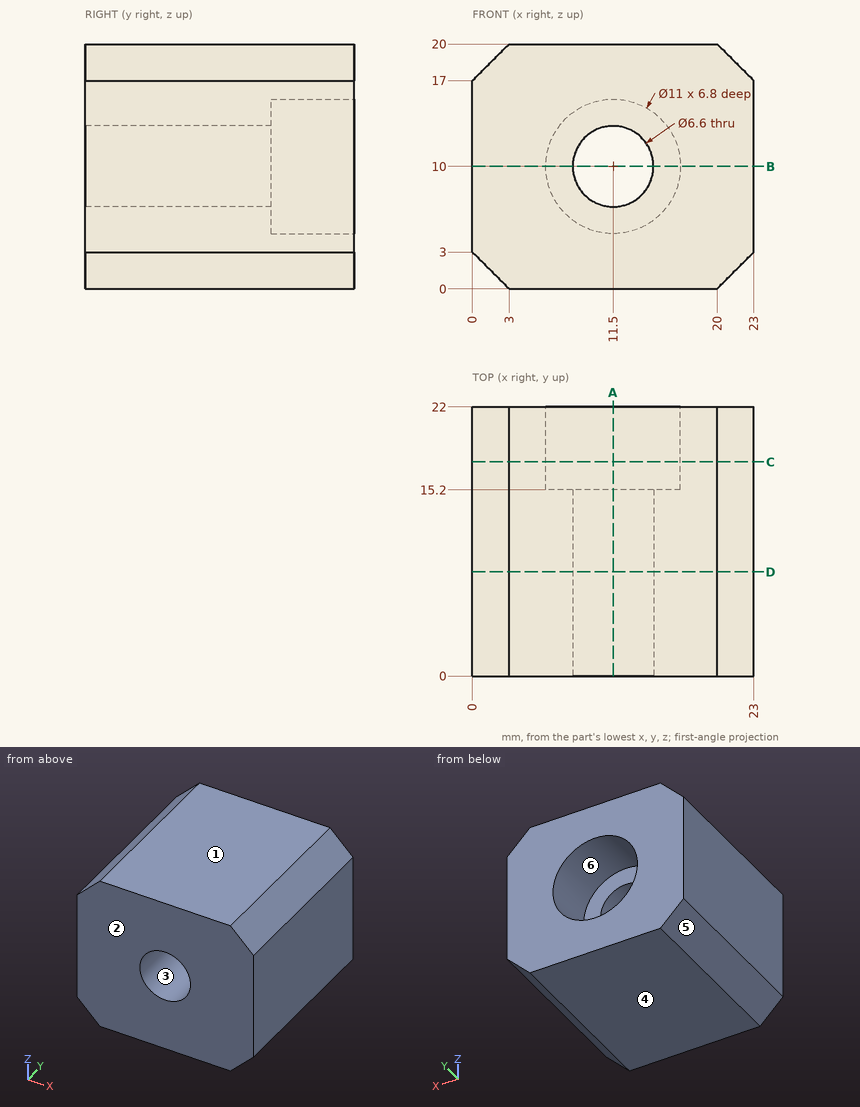
Can you work these out from the drawing? Everything is in mm from the part's minimum corner. A direction names the side the tool comes from. Round coordinates to 2 decimals unless told otherwise and drop trailing zeros. Write each loop counter-clockwise with the first axis right and the second up, starting at its lowest first coordinate (ties: lowest second). Pieces come first, ordered by that corner, then holes. Notation, with made-up numbers: (29.5, -6.5) - (52.5, -6.5) arc R18 ccw to (52.5, 15.5) - close; hole circle Ø5 at (-14, 24.5). An arc over 180 degrees is marked (long way). Put each result on its own line as item: value. Start each with the question number.
(1) I need wall thicknesses on probe 1 along X at (y, z) = (4.75, 10); probe 2 along Z at (x, y) = (11.5, 11.5); probe 3 along Z at (x, y) = (11.5, 16.75). Which ranges of each line are inside material? Lowest first, please.
(2) I want a section at A-A, the plane x = 11.5. Please give me the cut outline in (y, z), plus the area to 3 significant figures.
(3) I want a section at C-C, the plane y = 17.5. Please give me the cut outline in (x, z).
(4) Will these pins go through, and if not, where does the flat tip stop? pin 1 (3.5 mm diameter, centred on x = 13, z = 9, fed in from +Y); pin 2 (5.5 mm diameter, centred on x = 11.5, z = 10, fed in from -Y).
(5) I want a section at D-D, the plane y = 8.5. Please give me the cut outline in (x, z), plus the area to 3 significant figures.
(6) Thinking about a two-plate mould opening in Z: for the marked faces 1, 2, 3 and 4, which applies, released by +Z, released by -Z, zero draft, split by the parting line, or undercut?
(7) I want a section at B-B, the plane z = 10. Please give me the cut outline in (x, y), plus the area to 3 significant figures.
(8) For the marked faces 5 and 6, which set-ups out of +Z, -Z, +X, -X, +Y, -Y let a thin tool reach every point of the face, with its end or its side?
Here are the results:
1. probe 1: x = 0 to 8.2, 14.8 to 23
1. probe 2: z = 0 to 6.7, 13.3 to 20
1. probe 3: z = 0 to 4.5, 15.5 to 20
2. outline: (0, 0) - (22, 0) - (22, 4.5) - (15.2, 4.5) - (15.2, 6.7) - (0, 6.7) - close; (0, 13.3) - (15.2, 13.3) - (15.2, 15.5) - (22, 15.5) - (22, 20) - (0, 20) - close
2. area: 265 mm^2
3. outline: (0, 3) - (3, 0) - (20, 0) - (23, 3) - (23, 17) - (20, 20) - (3, 20) - (0, 17) - close; hole circle Ø11 at (11.5, 10)
4. pin 1: stops at y = 15.2
4. pin 2: passes through
5. outline: (0, 3) - (3, 0) - (20, 0) - (23, 3) - (23, 17) - (20, 20) - (3, 20) - (0, 17) - close; hole circle Ø6.6 at (11.5, 10)
5. area: 408 mm^2
6. face 1: released by +Z
6. face 2: zero draft
6. face 3: undercut
6. face 4: released by -Z
7. outline: (0, 0) - (8.2, 0) - (8.2, 15.2) - (6, 15.2) - (6, 22) - (0, 22) - close; (14.8, 0) - (23, 0) - (23, 22) - (17, 22) - (17, 15.2) - (14.8, 15.2) - close
7. area: 331 mm^2
8. face 5: -Z, -X, +Y, -Y
8. face 6: +Y
